The listing builds one solid part. Answer for the finished solid, in the listing's coordinates (mm). A direction names the side the tool comes from. Round coordinates to 2 decimals unless told otherwise and drop trailing zeros. Loops run counter-clockwise (first coordinate to the right, second up) from the corner with the lowest first, then second, coordinate; pieces in that order, holes last. Notation, with made-up numbers: (22, 49.5) - (62, 49.5) arc R13 ccw to (62, 74.5) - close; hole circle Ø7 at (-24, -0.75). An arc over 180 degrees is marked (long way). One line per question, with ' | ' between items. Start each with the question number.
from build123d import *

# Parameters (mm, degrees)
BASE_PLATE_DEPTH    = 32
FORK_ARM_DEPTH      = 16
HUB_SKETCH_R        = 44
HUB_88_DEPTH        = 56
KEYED_BORE_50_DEPTH = 56
PIN_HOLE_SKETCH_R   = 16
PIN_HOLES_32_DEPTH  = 255


with BuildPart() as part:
    # Base Plate Sketch → Base Plate (new body)
    with BuildSketch(Plane.XY):
        Polygon((0, 0), (83, 0), (83, 88), (-83, 88), (-83, 0), align=None)
    extrude(amount=-BASE_PLATE_DEPTH)

    # Fork Arm Sketch → Fork Arm (add)
    with BuildSketch(Plane(origin=(83, 0, 0), x_dir=(0, 0, -1), z_dir=(1, 0, 0))):
        with BuildLine():
            Line((32, 88), (77.221428654, 81.863206381))
            ThreePointArc((77.221428654, 81.863206381), (111.998506035, 44.336955652), (77.892381001, 6.199876056))
            Line((77.892381001, 6.199876056), (32, 0))
            Line((32, 0), (32, 88))
        make_face()
    fork_arm = extrude(amount=-FORK_ARM_DEPTH)

    # Fork Arm Mirror: Fork Arm across plane
    add(fork_arm.mirror(Plane(origin=(0, 0, 0), x_dir=(0, 0, 1), z_dir=(1, 0, 0))))

    # Hub Sketch → Hub Ø88 (add)
    with BuildSketch(Plane.XY):
        with Locations(Location((0, 44, 0), (0, 0, 270))):
            Circle(HUB_SKETCH_R)
    extrude(amount=HUB_88_DEPTH)

    # Keyed Bore Sketch → Keyed Bore Ø50 (cut)
    with BuildSketch(Plane.XY.offset(56)):
        with BuildLine():
            Line((24.494897428, 49), (29.494897428, 49))
            Line((29.494897428, 49), (29.494897428, 42))
            Line((29.494897428, 42), (24.919871589, 42))
            ThreePointArc((24.919871589, 42), (-24.954054766, 42.485024502), (24.494897428, 49))
        make_face()
    extrude(amount=-KEYED_BORE_50_DEPTH, mode=Mode.SUBTRACT)

    # Pin Hole Sketch → Pin Holes Ø32 (cut)
    with BuildSketch(Plane(origin=(83, 0, 0), x_dir=(0, 0, -1), z_dir=(1, 0, 0))):
        with Locations(Location((74, 44, 0), (0, 0, 180))):
            Circle(PIN_HOLE_SKETCH_R)
    extrude(amount=-PIN_HOLES_32_DEPTH, mode=Mode.SUBTRACT)


solid = part.part
(1) Find section B-B on y = 57. Write down the section's boundary in (x, z), plus the area to 3 significant figures.
(2) Each of these flat-tipped pins is pushed along its axis until it touches: P1, Ø2.5, axis at x = 27, z = 21, coming from the +Y side; P2, Ø4, axis at x = 61.5, y = 47, coming from the +Z side; P3, Ø7.5, axis at y = 46, z = 30.5, coming from the -X side. Where does it stop, or does it pass through?
(3) Find section A-A on z = 23. Write down the section's boundary in (x, y), plus the area to 3 significant figures.
(4) Determine the mould class of faces 1 (the flat face through (29.495, 46, 28)), 2 (the cylindrical face through (-16.852, 3.355, 27.608)), 3 (the flat face through (67, 45, -55)) for opening direction Y: pulls with the +Y half, pulls with the -Y half, needs draft (parallel to the pull), parting line crosses it, or undercut.
(5) A tool of negligible diameter and unlimited length cuts with its end or side. For faces 4 (the flat face through (-67, 45, -55)), 5 (the flat face through (-75.112, 84.975, -54.294)), 6 (the flat face through (3, 44, 0)), from which of +Z, -Z, +X, -X, +Y, -Y can it reach the whole face along a straight path? Write none if from no direction.
(6) Find section D-D on x = -7. Write down the section's boundary in (y, z), plus the area to 3 significant figures.
(7) Consider L1, parallel to X at y = 63, z = -62.5; L2, parallel to X at y = 44, z = 22; L3, parallel to Z at x = -28.5, y = 13. Determine where each line is inside the solid, lowest interval first.
(8) Find section C-C on z = -87.5. Write down the section's boundary in (x, y).
Answer below:
1) outline: (-83, -109.71) - (-67, -109.71) - (-67, -83.33) - (-83, -83.33) - close; (-83, -64.67) - (-67, -64.67) - (-67, -32) - (67, -32) - (67, -64.67) - (83, -64.67) - (83, 0) - (42.04, 0) - (42.04, 56) - (21.35, 56) - (21.35, 0) - (-21.35, 0) - (-21.35, 56) - (-42.04, 56) - (-42.04, 0) - (-83, 0) - close; (67, -109.71) - (83, -109.71) - (83, -83.33) - (67, -83.33) - close | area: 9,520 mm2
2) P1: y = 79.68 | P2: z = 0 | P3: x = -44
3) outline: circle Ø88 at (0, 44); hole (24.49, 49) arc R25 ccw (long way) to (24.92, 42) - (29.49, 42) - (29.49, 49) - close | area: 4,090 mm2
4) face 1: undercut | face 2: parting line crosses it | face 3: needs draft
5) face 4: -Z, +Y, -Y | face 5: -Z, +X, -X, +Y | face 6: +Z
6) outline: (0, -32) - (88, -32) - (88, 0) - (87.44, 0) - (87.44, 56) - (68, 56) - (68, 0) - (20, 0) - (20, 56) - (0.56, 56) - (0.56, 0) - (0, 0) - close | area: 4,990 mm2
7) L1: -83 to -67, 67 to 83 | L2: -44 to -25, 29.49 to 44 | L3: -32 to 56
8) outline: (-83, 8.48) - (-67, 8.48) - (-67, 35.41) - (-83, 35.41) - close; (-83, 52.59) - (-67, 52.59) - (-67, 79.52) - (-83, 79.52) - close; (67, 8.48) - (83, 8.48) - (83, 35.41) - (67, 35.41) - close; (67, 52.59) - (83, 52.59) - (83, 79.52) - (67, 79.52) - close
